The listing builds one solid part. Answer for the finished solid, in the listing's coordinates (mm). A direction names the side the tool comes from. Round coordinates to 2 decimals unless told otherwise and drop trailing zeros. Loops run counter-clockwise (first coordinate to the right, second up) from the corner with the lowest first, then second, coordinate; pieces in that order, holes last. Notation, with made-up numbers: (38, 83) -> (57, 83) arc R20 cw to (57, 93) -> close; hole circle Ø10 at (-11, -32.75). An arc over 180 degrees is marked (long way). Use a Markdown table: item, result. Add a question column.
Q1. Section A-A on x = 26.5 is taken. Give the vertices of the cut face in (y, z).
Q2. Section B-B on z = 30 is taken. Give the vertices of the cut face in (x, y), then the cut area to 3 significant figures.
Q3. Section C-C on z = 10 is taken. Give the vertices of the cut face in (x, y), then the cut area to 3 significant figures.
Q4. Consider line 1 (Y direction, x = 0, z = 7.25); line 2 (Z direction, x = 110, y = -4); line 3 (X direction, y = -18.5, z = 18). Determine where each line is inside the solid, lowest interval first.
Q5. Section D-D on y = -17 is taken. Give the vertices of the cut face in (x, z), then the cut area to 3 significant figures.
Q6. Which of the six approach directions +Z, -Z, +X, -X, +Y, -Y give full straight-line access (tool end or side, diameter ignored) to faces 1 (the cylindrical face through (139.745, -14.65, 26.095)), 2 (the flat face through (9, 2, 46)), 3 (the flat face through (51, 5, 60))?
Q7. For a pull along Z with two mould halves and no side action, classify faces 4 (the cylindrical face through (137.266, -14.65, 26.42)), 5 (the cylindrical face through (-7.3, -6.834, 6.902)), 6 (the flat face through (51, 5, 0)) as released by +Z, released by -Z, zero draft, split by the parting line, or undercut.
Q8. Given pin 1 Ø1.5 at (y, z) = (-27.5, 53.5) entering from +X; pin 2 Ø22 at (x, y) = (24.5, -1.5) entering from -Z; pin 3 Ø5.5 at (x, y) = (0, 0) entering from +Z; pin 4 Ø8 at (y, z) = (4, 25.5) entering from -X, each flat-ended and moving along its own axis, determine where each tip first touches the part or whether it passes through.
from build123d import *

# Parameters (mm, degrees)
SKETCH1_R               = 10
SKETCH1_R_2             = 3
BOSS_EXTRUDE1_DEPTH     = 60
BOSS_EXTRUDE2_START     = -60
BOSS_EXTRUDE2_DEPTH     = 60
CUT_EXTRUDE1_DEPTH      = 127.885775404
CUT_EXTRUDE1_DEPTH_BACK = 127.885775404
SKETCH4_W               = 97.330885133
SKETCH4_H               = 32
SKETCH5_R               = 30
SKETCH5_R_2             = 27.5
BOSS_EXTRUDE3_DEPTH     = 50
CUT_EXTRUDE2_DEPTH      = 161.312195419
CUT_EXTRUDE2_DEPTH_BACK = 161.312195419
SKETCH6_R               = 27.5


with BuildPart() as part:
    # Sketch1 → Boss-Extrude1 (new body)
    with BuildSketch(Plane.XY):
        Circle(SKETCH1_R)
        Circle(SKETCH1_R_2, mode=Mode.SUBTRACT)
    extrude(amount=BOSS_EXTRUDE1_DEPTH)

    # Sketch3 → Boss-Extrude2 (add)
    with BuildSketch(Plane.XY.offset(60).offset(BOSS_EXTRUDE2_START)):
        with BuildLine():
            Line((0, 10), (110, 10))
            Line((110, 10), (110, 0))
            Line((110, 0), (10, 0))
            ThreePointArc((10, 0), (7.071067812, 7.071067812), (0, 10))
        make_face()
    extrude(amount=BOSS_EXTRUDE2_DEPTH)

    # Sketch4 → Cut-Extrude1 (cut, two sides: drawn at the far end of the back side and taken through both)
    with BuildSketch(Plane(origin=(0, 10, 0), x_dir=(1, 0, 0), z_dir=(0, 1, 0)).offset(-CUT_EXTRUDE1_DEPTH_BACK)):
        with Locations((-8.665442567, -30)):
            Rectangle(SKETCH4_W, SKETCH4_H)
    extrude(amount=CUT_EXTRUDE1_DEPTH + CUT_EXTRUDE1_DEPTH_BACK, mode=Mode.SUBTRACT)

    # Sketch5 → Boss-Extrude3 (add)
    with BuildSketch(Plane(origin=(0, 10, 0), x_dir=(1, 0, 0), z_dir=(0, 1, 0))):
        with Locations(Location((110, -30, 0), (0, 0, 270))):
            Circle(SKETCH5_R)
        with Locations(Location((110, -30, 0), (0, 0, 270))):
            Circle(SKETCH5_R_2, mode=Mode.SUBTRACT)
    extrude(amount=-BOSS_EXTRUDE3_DEPTH)

    # Sketch6 → Cut-Extrude2 (cut, two sides: drawn at the far end of the back side and taken through both)
    with BuildSketch(Plane(origin=(0, 10, 0), x_dir=(1, 0, 0), z_dir=(0, 1, 0)).offset(-CUT_EXTRUDE2_DEPTH_BACK)):
        with Locations(Location((110, -30, 0), (0, 0, 270))):
            Circle(SKETCH6_R)
    extrude(amount=CUT_EXTRUDE2_DEPTH + CUT_EXTRUDE2_DEPTH_BACK, mode=Mode.SUBTRACT)


solid = part.part
Checked values:
| question | item | result |
|---|---|---|
| 1 | outline | (0, 0) -> (10, 0) -> (10, 14) -> (0, 14) -> close; (0, 46) -> (10, 46) -> (10, 60) -> (0, 60) -> close |
| 2 | outline | (40, 0) -> (80, 0) -> (80, -40) -> (82.5, -40) -> (82.5, 10) -> (40, 10) -> close; (137.5, -40) -> (140, -40) -> (140, 10) -> (137.5, 10) -> close |
| 2 | area | 650 mm2 |
| 3 | outline | (0, 10) arc R10 ccw (long way) to (10, 0) -> (87.64, 0) -> (87.64, -40) -> (91.13, -40) -> (91.13, 10) -> close; (128.87, -40) -> (132.36, -40) -> (132.36, 10) -> (128.87, 10) -> close; hole circle Ø6 at (0, 0) |
| 3 | area | 1,430 mm2 |
| 4 | line 1 | y = -10 to -3, 3 to 10 |
| 4 | line 2 | z = 0 to 2.5, 57.5 to 60 |
| 4 | line 3 | x = 82.5 to 85.26, 134.74 to 137.5 |
| 5 | outline | circle Ø60 at (110, 30); hole circle Ø55 at (110, 30) |
| 5 | area | 452 mm2 |
| 6 | face 1 | -Y |
| 6 | face 2 | -X, +Y, -Y |
| 6 | face 3 | +Z, +X, -X, +Y, -Y |
| 7 | face 4 | undercut |
| 7 | face 5 | zero draft |
| 7 | face 6 | released by -Z |
| 8 | pin 1 | stops at x = 129.56 |
| 8 | pin 2 | stops at z = 0 |
| 8 | pin 3 | passes through |
| 8 | pin 4 | stops at x = 40 |
